Model file for the job. Use its own axes, mm. Face numbers are marked on the shaded views. A direction names the side the tool comes from. Round coordinates to 2 decimals unless told otherwise and drop trailing zeros. Loops run counter-clockwise (first coordinate to the right, second up) from the corner with the lowest first, then second, coordinate; pieces in that order, holes last. Notation, with made-up numbers: M 17.25,42 L 32.25,42 A25 cw 32.25,68 Z; hole C -25.5,-9.5 d4. An arc over 180 degrees is marked long. Answer in a Markdown table with one row per item.
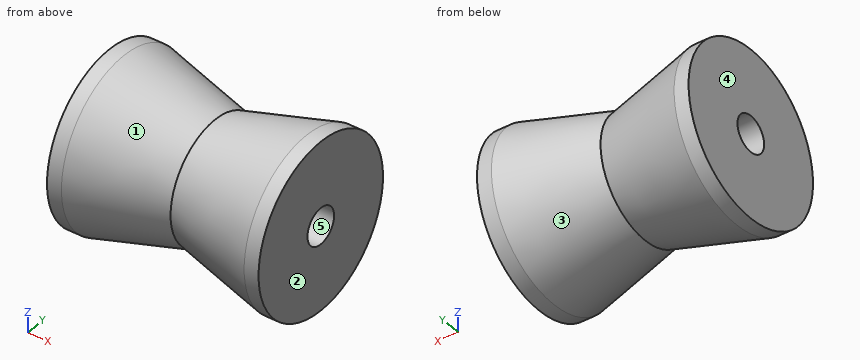
from build123d import *


with BuildPart() as part:
    # Roller Profile Sketch → Roller Body Revolve (revolve)
    with BuildSketch(Plane.XY, mode=Mode.PRIVATE) as roller_body_revolve_sk:
        Polygon((0, 50), (-38, 60), (-44, 60), (-44, 32.5), (44, 32.5), (44, 60), (38, 60), align=None)
    revolve(roller_body_revolve_sk.sketch.rotate(Axis((-44, 25, 0), (1, 0, 0)), 90), axis=Axis((-44, 25, 0), (1, 0, 0)))


solid = part.part
1. Tool access for the marked faces 1 and 2: list every direction of +Z, -Z, +X, -X, +Y, -Y with a clear straight run to the whole face (end or side of a thin tool).
Verdict:
| item | result |
|---|---|
| face 1 | none |
| face 2 | +Z, -Z, +X, +Y, -Y |
2. Saw through at A-A (y = 25). Write the cut outline in (x, z), and give its area (3 significant figures).
Verdict:
| item | result |
|---|---|
| outline | M -44,-35 L -38,-35 L 0,-25 L 38,-35 L 44,-35 L 44,-7.5 L -44,-7.5 Z; M -44,7.5 L 44,7.5 L 44,35 L 38,35 L 0,25 L -38,35 L -44,35 Z |
| area | 4,080 mm² |
3. Saw through at C-C (x = 20.5). Write the cut outline in (y, z).
Verdict:
| item | result |
|---|---|
| outline | C 25,0 d60.79; hole C 25,0 d15 |
4. Wall check: probe 1 along Y at (x, z) = (-12.5, -1.5); probe 2 along Y at (x, z) = (30, 0.5); probe 3 along Z at (x, y) = (35, 22). Give the ranges that are in metal, low to high.
Verdict:
| item | result |
|---|---|
| probe 1 | y = -3.25 to 17.65, 32.35 to 53.25 |
| probe 2 | y = -7.89 to 17.52, 32.48 to 57.89 |
| probe 3 | z = -34.08 to -6.87, 6.87 to 34.08 |
5. Saw through at B-B (z = 0). Write the cut outline in (x, y).
Verdict:
| item | result |
|---|---|
| outline | M -44,-10 L -38,-10 L 0,0 L 38,-10 L 44,-10 L 44,17.5 L -44,17.5 Z; M -44,32.5 L 44,32.5 L 44,60 L 38,60 L 0,50 L -38,60 L -44,60 Z |
6. Mould opens along Z. For the marked faces 3, 4 and 5 say: +Z half, -Z half, draft (parallel to the pull), parting line (faces both ways), or undercut.
Verdict:
| item | result |
|---|---|
| face 3 | parting line |
| face 4 | draft |
| face 5 | undercut |
7. Pin check, flat tips, straight feed: pin 1 (1.5 mm diameter, centred on x = -10, z = 20.5, fed in from +Y); pin 2 (6 mm diameter, centred on x = 11, y = 35.5, fed in from +Z); pin 3 (8 mm diameter, centred on x = 22.5, y = 11.5, fed in from +Z). Stop position of each tip, or through.
Verdict:
| item | result |
|---|---|
| pin 1 | stops at y = 44.37 |
| pin 2 | stops at z = 27.19 |
| pin 3 | stops at z = 29.83 |
8. Saw through at D-D (x = 6). Write the cut outline in (y, z).
Verdict:
| item | result |
|---|---|
| outline | C 25,0 d53.16; hole C 25,0 d15 |
